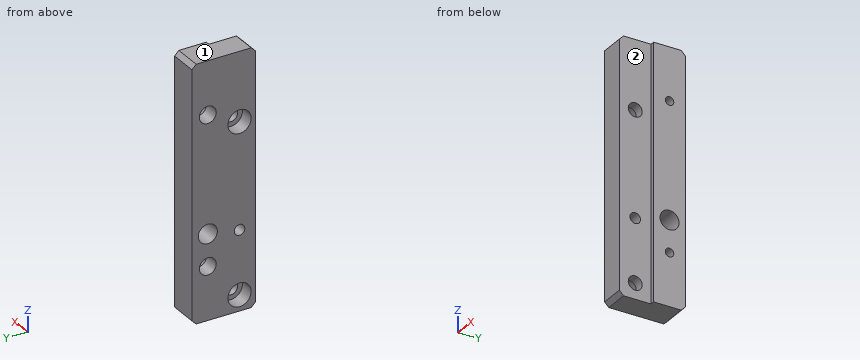
```python
from build123d import *

# Parameters (mm, degrees)
SKETCH1_W                                            = 120
SKETCH1_H                                            = 30
BOSS_EXTRUDE1_DEPTH                                  = 13.4
SKETCH2_W                                            = 120
SKETCH2_H                                            = 15
CUT_EXTRUDE1_DEPTH                                   = 2
HOLE1_AT_2_COUNT                                     = 2
HOLE1_AT_2_PITCH                                     = 70
M8_CLEARANCE_HOLE1_D                                 = 9
CHAMFER1_SIZE                                        = 2
CBORE_FOR_M6_HEXAGON_SOCKET_HEAD_CAP_SCR_D           = 6.6
CBORE_FOR_M6_HEXAGON_SOCKET_HEAD_CAP_SCR_CBORE_D     = 11
CBORE_FOR_M6_HEXAGON_SOCKET_HEAD_CAP_SCR_CBORE_DEPTH = 6.8
F_5_0MM_BLIND_HOLE_1_D                               = 5


with BuildPart() as part:
    # Sketch1 → Boss-Extrude1 (new body)
    with BuildSketch(Plane(origin=(0, 0, 0), x_dir=(0, 0, -1), z_dir=(1, 0, 0))):
        Rectangle(SKETCH1_W, SKETCH1_H)
    extrude(amount=BOSS_EXTRUDE1_DEPTH)

    # Sketch2 → Cut-Extrude1 (cut)
    with BuildSketch(Plane(origin=(13.4, 0, 0), x_dir=(0, 0, -1), z_dir=(1, 0, 0))):
        with Locations((0, -7.5)):
            Rectangle(SKETCH2_W, SKETCH2_H)
    extrude(amount=-CUT_EXTRUDE1_DEPTH, mode=Mode.SUBTRACT)

    # Sketch4 → Hole1 (revolve, cut)
    with BuildSketch(Plane(origin=(0, 7.5, 35), x_dir=(0, 0, 1), z_dir=(0, 1, 0))):
        Polygon((0, 0), (0, 20), (2, 20), (2, 8.701721238), (4, 7.5), (4, 0), align=None)
    hole1 = revolve(axis=Axis((-6.130023899, 7.5, 35), (1, 0, 0)), mode=Mode.SUBTRACT)

    # Hole1 at 2: Hole1 ×2
    with Locations(*[(0, 0, -i * HOLE1_AT_2_PITCH) for i in range(1, HOLE1_AT_2_COUNT)]):
        add(hole1, mode=Mode.SUBTRACT)

    # M8 Clearance Hole1 (through all)
    with Locations(Plane(origin=(13.4, 0, 0), x_dir=(0, 0, -1), z_dir=(1, 0, 0))):
        with Locations((20, 7.5)):
            Hole(M8_CLEARANCE_HOLE1_D / 2)

    # Chamfer1
    chamfer1_edges = [part.edges().sort_by_distance(p)[0] for p in [
        (5.7, -15, -60),
        (5.7, -15, 60),
        (6.7, 15, 60),
        (6.7, 15, -60),
    ]]
    chamfer(chamfer1_edges, length=CHAMFER1_SIZE)

    # CBORE for M6 Hexagon socket head cap screws1 (through all)
    with Locations(Plane.ZY):
        with Locations((-52.5, -7.5), (27.5, -7.5)):
            CounterBoreHole(CBORE_FOR_M6_HEXAGON_SOCKET_HEAD_CAP_SCR_D / 2, CBORE_FOR_M6_HEXAGON_SOCKET_HEAD_CAP_SCR_CBORE_D / 2, CBORE_FOR_M6_HEXAGON_SOCKET_HEAD_CAP_SCR_CBORE_DEPTH)

    # Ø5.0mm blind hole 1 (through all)
    with Locations(Plane.ZY):
        with Locations((-22.5, -7.5)):
            Hole(F_5_0MM_BLIND_HOLE_1_D / 2)


solid = part.part
```
Can you work these out from the model? Positions are in its coordinate system, mm. Face numbers are marked on the shaded views. A direction names the side the tool comes from. Give positions to 0.01 mm unless a question says otherwise; leave off trailing zeros. Loops run counter-clockwise (first coordinate to the right, second up) from the corner with the lowest first, then second, coordinate; pieces in that order, holes last. Notation, with made-up numbers: M -14,0 L 37,0 A22 cw 37,33 Z; hole C 14.25,3.25 d1. An arc over 180 degrees is marked long. Answer in a Markdown table with one row per item.
1. Suppose I cut it at C-C on x = 5. Write out the boundary of the cut face in (y, z).
Taken from the geometry:
| item | result |
|---|---|
| outline | M -15,-58 L -13,-60 L 13,-60 L 15,-58 L 15,58 L 13,60 L -13,60 L -15,58 Z; hole C -7.5,-52.5 d11; hole C -7.5,27.5 d11; hole C -7.5,-22.5 d5; hole C 7.5,-20 d9; hole C 7.5,-35 d8; hole C 7.5,35 d8 |
2. Which directions (+Z, -Z, +X, -X, +Y, -Y) give clear straight access to the entire face, cutting with the end or side of a thin tool? Please do the marked faces 1 and 2.
Taken from the geometry:
| item | result |
|---|---|
| face 1 | +Z, +X, -X, +Y, -Y |
| face 2 | +Z, -Z, +X, -Y |
3. Suppose I cut it at D-D on z = -22.5. Write out the boundary of the cut face in (x, y), plus the area to 3 significant figures.
Taken from the geometry:
| item | result |
|---|---|
| outline | M 0,-15 L 11.4,-15 L 11.4,-10 L 0,-10 Z; M 0,-5 L 11.4,-5 L 11.4,0 L 13.4,0 L 13.4,3.76 L 0,3.76 Z; M 0,11.24 L 13.4,11.24 L 13.4,15 L 0,15 Z |
| area | 215 mm² |
4. If I drill on line 1 along Y through (x, z) = (8.75, -35); line 2 along Y through (x, z) = (11.5, -35); line 3 along X through (y, z) = (-10.5, 33.5), over which ranges is the centre line in solid material (lowest first)?
Taken from the geometry:
| item | result |
|---|---|
| line 1 | y = -15 to 5.5, 9.5 to 15 |
| line 2 | y = 0 to 5.5, 9.5 to 15 |
| line 3 | x = 0 to 11.4 |
5. For pin 1 Ø1 at (x, z) = (12, 8) entering from -Y; pin 2 Ø4.5 at (y, z) = (7.5, 35) entering from +X; pin 3 Ø8 at (y, z) = (-6.5, 4) entering from +X; pin 4 Ø9 at (y, z) = (-7, -53) entering from -X, each with a flat end and sliding along its axis, tell me the tip position at first contact or that it passes through.
Taken from the geometry:
| item | result |
|---|---|
| pin 1 | stops at y = 0 |
| pin 2 | stops at x = 13.4 |
| pin 3 | stops at x = 11.4 |
| pin 4 | stops at x = 6.8 |
6. Suppose I cut it at B-B on z = -52.5. Write out the boundary of the cut face in (x, y).
Taken from the geometry:
| item | result |
|---|---|
| outline | M 0,-15 L 11.4,-15 L 11.4,-10.8 L 6.8,-10.8 L 6.8,-13 L 0,-13 Z; M 0,-2 L 6.8,-2 L 6.8,-4.2 L 11.4,-4.2 L 11.4,0 L 13.4,0 L 13.4,15 L 0,15 Z |
7. Suppose I cut it at A-A on y = -7.5. Write out the boundary of the cut face in (x, z), plus the area to 3 significant figures.
Taken from the geometry:
| item | result |
|---|---|
| outline | M 0,-60 L 11.4,-60 L 11.4,-55.8 L 6.8,-55.8 L 6.8,-58 L 0,-58 Z; M 0,-47 L 6.8,-47 L 6.8,-49.2 L 11.4,-49.2 L 11.4,-25 L 0,-25 Z; M 0,-20 L 11.4,-20 L 11.4,24.2 L 6.8,24.2 L 6.8,22 L 0,22 Z; M 0,33 L 6.8,33 L 6.8,30.8 L 11.4,30.8 L 11.4,60 L 0,60 Z |
| area | 1,100 mm² |
